Drawing for the job (mm, zero at the part's lowest x, y, z). A direction names the side the tool comes from. Round coordinates to 2 decimals unless told otherwise and drop trailing zeros. Order: outer loops, then holes, each group sorted by start corner. A loop starts at its lowest first (then second) coordinate and runs counter-clockwise, first axis right, second up. Notation, with made-up numbers: (14, 66.25) - (42, 66.25) arc R37 ccw to (42, 102.25) - close; hole circle Ø6 at (86.5, 80.25). An arc over 180 degrees is marked (long way). Answer as a JSON object with one key per item and string values.
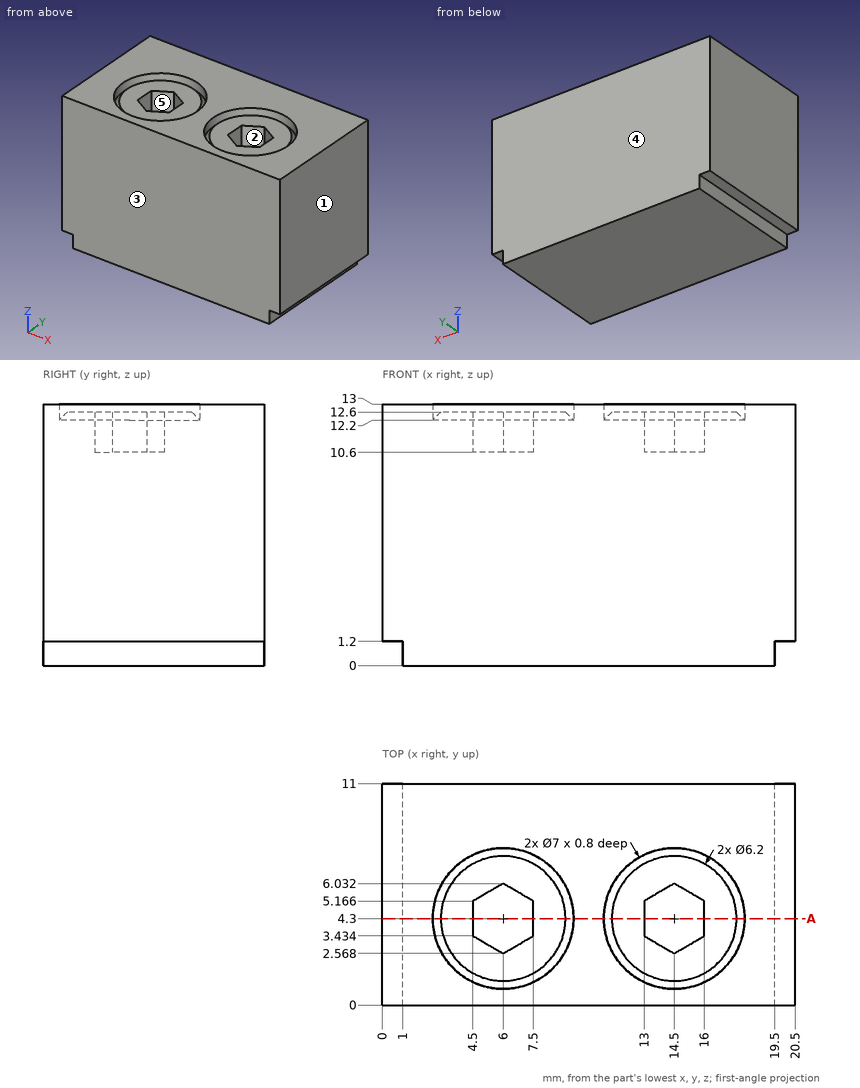
Item 1: Two-plate mould, pull along X, no slides. Class the marked faces 1, 2 and 3: pulls with the +X half, pulls with the -X half, needs draft (parallel to the pull), parting line crosses it, or undercut.
Taken from the geometry:
{"face 1": "pulls with the +X half", "face 2": "undercut", "face 3": "needs draft"}
Item 2: Probe L1, parallel to X at y = 4.3, z = 12.8; L2, parallel to Y at x = 14.5, z = 12.65; L3, parallel to Z at x = 5.75, y = 3.5. List the from-to ranges inside material, lowest first. Write a range as from..to.
Taken from the geometry:
{"L1": "0..2.5, 9.5..11, 18..20.5", "L2": "0..0.8, 7.8..11", "L3": "0..10.6"}
Item 3: Cut at A-A (y = 4.3). Write the cut outline in (x, z).
Taken from the geometry:
{"outline": "(0, 1.2) - (1, 1.2) - (1, 0) - (19.5, 0) - (19.5, 1.2) - (20.5, 1.2) - (20.5, 13) - (18, 13) - (18, 12.2) - (17.6, 12.6) - (16, 12.6) - (16, 10.6) - (13, 10.6) - (13, 12.6) - (11.4, 12.6) - (11, 12.2) - (11, 13) - (9.5, 13) - (9.5, 12.2) - (9.1, 12.6) - (7.5, 12.6) - (7.5, 10.6) - (4.5, 10.6) - (4.5, 12.6) - (2.9, 12.6) - (2.5, 12.2) - (2.5, 13) - (0, 13) - close"}
Item 4: Drop flat-ended pins along their axis: P1, Ø1.9, axis at x = 16, y = 5, coming from the +Z side; P2, Ø0.8, axis at x = 20, y = 4, coming from the -Z side; P3, Ø1.3, axis at y = 5.5, z = 0.5, coming from the +X side. Give the stop position or say it passes through.
Taken from the geometry:
{"P1": "z = 12.6", "P2": "z = 1.2", "P3": "x = 19.5"}
Item 5: Tool access for the marked faces 4 and 5: list every direction of +Z, -Z, +X, -X, +Y, -Y with a clear straight run to the whole face (end or side of a thin tool).
Taken from the geometry:
{"face 4": "+Z, -Z, +X, -X, +Y", "face 5": "+Z"}
